Can you work these out from the drawing? Everything is in mm from the part's minimum corner. Round coordinates to 2 decimals unless told otherwise and drop trailing zeros. Write each loop counter-clockwise with the first axis right and the second up, starting at its lowest first coordinate (ties: lowest second). Pieces come first, ordered by that corner, then holes. Notation, with made-up numbers: (54.5, 57.5) -> (104.5, 57.5) arc R22 ccw to (104.5, 71.5) -> close; hole circle Ø3 at (-11.5, 32.5). An arc over 180 degrees is marked (long way). One line per question, with ' | ' between items. Start each with the question number.
1. If I drill on line 1 along Y through (x, z) = (15.25, 3.05); line 2 along X through (y, z) = (59, 3.4); line 3 along Z through (x, y) = (12.5, 150.5), over which ranges is the centre line in solid material (lowest first)? Write a range as [from, to].
2. For pin 1 Ø0.9 at (x, z) = (18.5, 3) entering from -Y; pin 2 Ø4 at (x, y) = (24.5, 121) entering from -Z; pin 3 Ø1.5 at (x, z) = (21.5, 1) entering from -Y; pin 4 Ø3 at (x, z) = (3.5, 3.5) entering from -Y, each with a flat end and sliding along its axis, tell me the tip position at first contact or that it passes through.
3. Imagine slicing it at B-B, the plane y = 63. List the corners of the cut face in (x, z) for me.
4. Thinking about a two-plate mould opening in Y: for the marked faces 1 and 2, which applies, released by +Y, released by -Y, zero draft, split by the parting line, or undercut?
5. Imagine slicing it at C-C, the plane x = 15. List the corners of the cut face in (y, z) for me.
6. Imagine slicing it at A-A, the plane z = 2.8. List the corners of the cut face in (x, y) for me.
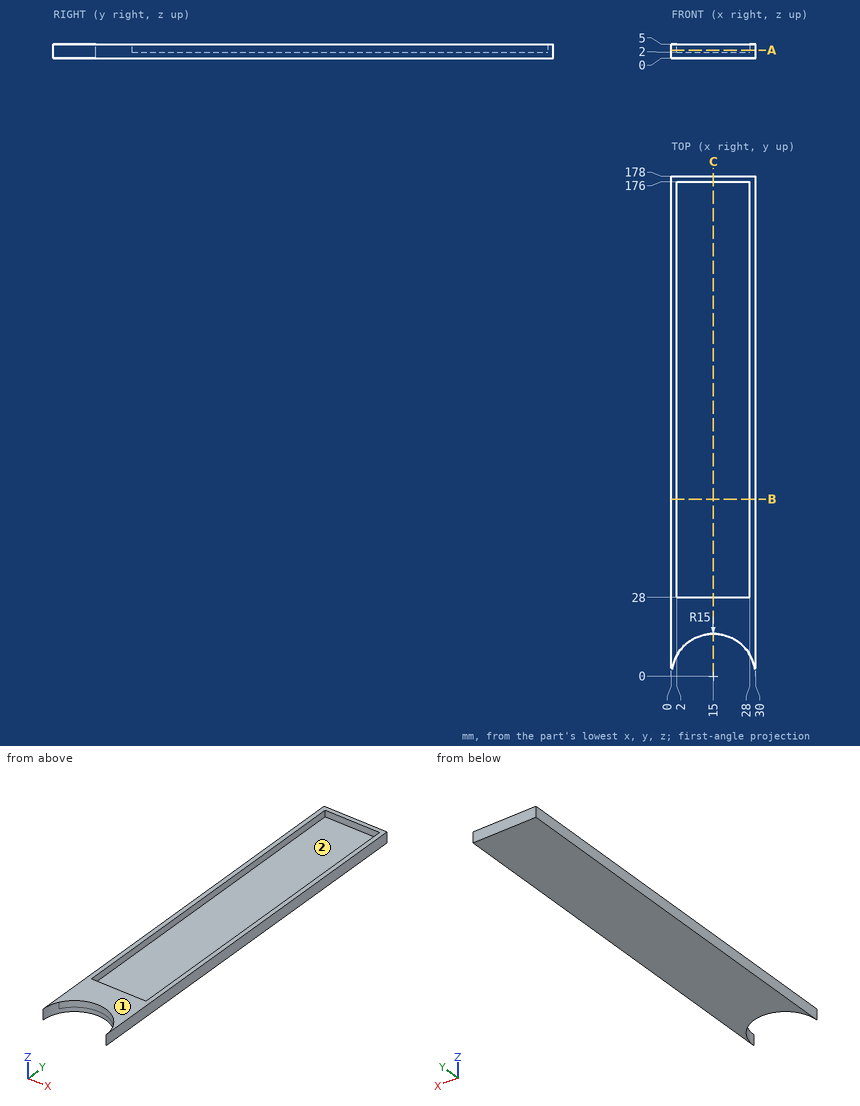
Geometry results:
1) line 1: y = [15, 28], [176, 178] | line 2: x = [0, 2], [28, 30] | line 3: z = [0, 2]
2) pin 1: stops at y = 14.47 | pin 2: stops at z = 0 | pin 3: stops at y = 13.13 | pin 4: stops at y = 7.48
3) outline: (0, 0) -> (30, 0) -> (30, 5) -> (28, 5) -> (28, 2) -> (2, 2) -> (2, 5) -> (0, 5) -> close
4) face 1: zero draft | face 2: undercut
5) outline: (15, 0) -> (178, 0) -> (178, 5) -> (176, 5) -> (176, 2) -> (28, 2) -> (28, 5) -> (15, 5) -> close
6) outline: (0, 0) arc R15 cw to (30, 0) -> (30, 178) -> (0, 178) -> close; hole (2, 28) -> (28, 28) -> (28, 176) -> (2, 176) -> close
